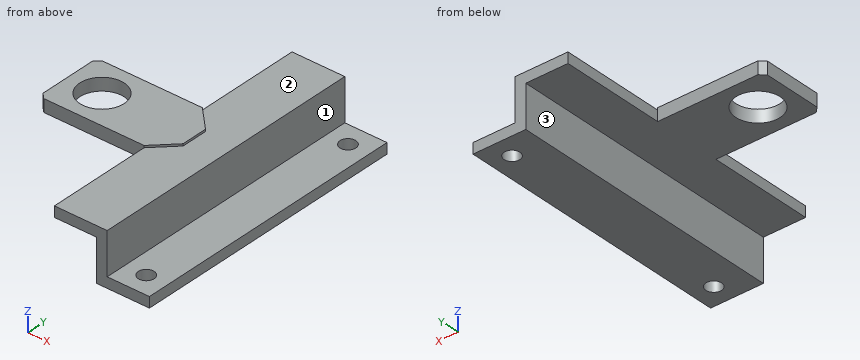
```python
from build123d import *

# Parameters (mm, degrees)
SKETCH_1_R          = 21
EXTRUDE_1_DEPTH     = 12
CHAMFER_1_SIZE      = 5
CHAMFER_2_SIZE      = 20
EXTRUDE_2_DEPTH     = 10
SKETCH_4_W          = 10
SKETCH_4_H          = 265
EXTRUDE_3_DEPTH     = 50
SKETCH_6_W          = 50
SKETCH_6_H          = 265
EXTRUDE_4_DEPTH     = 10
SKETCH_7_R          = 7.5
CUT_EXTRUDE_1_DEPTH = 211.063085762


with BuildPart() as part:
    # 草图1 → 凸台-拉伸1 (new body)
    with BuildSketch(Plane.XY):
        Polygon((32.5, 32.5), (87.5, 32.5), (87.5, -32.5), (32.5, -32.5), (-32.5, -32.5), (-32.5, 32.5), align=None)
        Circle(SKETCH_1_R, mode=Mode.SUBTRACT)
    extrude(amount=EXTRUDE_1_DEPTH)

    # 倒角1
    chamfer_1_edges = [part.edges().sort_by_distance(p)[0] for p in [
        (-32.5, -32.5, 6),
        (-32.5, 32.5, 6),
    ]]
    chamfer(chamfer_1_edges, length=CHAMFER_1_SIZE)

    # 倒角2
    chamfer_2_edges = [part.edges().sort_by_distance(p)[0] for p in [
        (87.5, 32.5, 6),
        (87.5, -32.5, 6),
    ]]
    chamfer(chamfer_2_edges, length=CHAMFER_2_SIZE)

    # 草图3 → 凸台-拉伸2 (add)
    with BuildSketch(Plane(origin=(0, 0, 0), x_dir=(-1, 0, 0), z_dir=(0, 0, -1))):
        Polygon((-67.5, 32.5), (-87.5, 12.5), (-87.5, -12.5), (-67.5, -32.5), (-67.5, -132.5), (-117.5, -132.5), (-117.5, 132.5), (-67.5, 132.5), align=None)
    extrude(amount=-EXTRUDE_2_DEPTH)

    # 草图4 → 凸台-拉伸3 (add)
    with BuildSketch(Plane.XY.offset(10)):
        with Locations((112.5, 0)):
            Rectangle(SKETCH_4_W, SKETCH_4_H)
    extrude(amount=-EXTRUDE_3_DEPTH)

    # 草图6 → 凸台-拉伸4 (add)
    with BuildSketch(Plane(origin=(0, 0, -40), x_dir=(-1, 0, 0), z_dir=(0, 0, -1))):
        with Locations((-132.5, 0)):
            Rectangle(SKETCH_6_W, SKETCH_6_H)
    extrude(amount=-EXTRUDE_4_DEPTH)

    # 草图7 → 切除-拉伸1 (cut, through all)
    with BuildSketch(Plane.XY.offset(-30)):
        with Locations((137.5, 112.5)):
            Circle(SKETCH_7_R)
        with Locations((137.5, -112.5)):
            Circle(SKETCH_7_R)
    extrude(amount=-CUT_EXTRUDE_1_DEPTH, mode=Mode.SUBTRACT)


solid = part.part
```
The listing builds one solid part. Answer for the finished solid, in the listing's coordinates (mm). Face numbers are marked on the shaded views. A direction names the side the tool comes from. Round coordinates to 2 decimals unless told otherwise and drop trailing zeros. Order: outer loops, then holes, each group sorted by start corner. A loop starts at its lowest first (then second) coordinate and runs counter-clockwise, first axis right, second up. Notation, with made-up numbers: (61, 49.25) - (68, 49.25) arc R4 cw to (68, 56.25) - close; hole circle Ø1 at (-22, 5.5). An arc over 180 degrees is marked (long way). Put each result on its own line as item: value. Start each with the question number.
(1) Find section A-A (y = 112.5). Give the vertices of the cut face in (x, z).
(2) Find section D-D (y = 0). Give the vertices of the cut face in (x, z), plus the area to 3 significant figures.
(3) Given P1, Ø6, axis at x = 31.5, z = 7, coming from the +Y side; P2, Ø12, axis at y = 96, z = -2.5, coming from the -X side; P3, Ø3.5, axis at x = 15.5, z = 6.5, coming from the -Y side; P4, Ø25, axis at x = 0, y = 0, coming from the -Z side, each flat-ended and moving along its own axis, determine where each tip first touches the part or whether it passes through.
(4) Find section C-C (x = 80). Give the vertices of the cut face in (y, z), plus the area to 3 significant figures.
(5) For the marked faces 1, 2 and 3, determine the directions among +Z, -Z, +X, -X, +Y, -Y from which every point of the face is accessible in a straight line to the end or side of a thin tool.
(6) Straight lines are drawn through the part: probe 1 along Y at (x, z) = (137, -32); probe 2 along Y at (x, z) = (0, 5); probe 3 along Z at (x, y) = (110.5, 117). For each, find the intervals that lie inside material, in ascending order. Write a range as from..to.
(7) Find section B-B (z = 7). Give the vertices of the cut face in (x, y).
Reply:
1. outline: (67.5, 0) - (107.5, 0) - (107.5, -40) - (130, -40) - (130, -30) - (117.5, -30) - (117.5, 10) - (67.5, 10) - close; (145, -40) - (157.5, -40) - (157.5, -30) - (145, -30) - close
2. outline: (-32.5, 0) - (-21, 0) - (-21, 12) - (-32.5, 12) - close; (21, 0) - (107.5, 0) - (107.5, -40) - (157.5, -40) - (157.5, -30) - (117.5, -30) - (117.5, 10) - (87.5, 10) - (87.5, 12) - (21, 12) - close
2. area: 2,040 mm^2
3. P1: y = 32.5
3. P2: x = 67.5
3. P3: y = -32.5
3. P4: through
4. outline: (-132.5, 0) - (132.5, 0) - (132.5, 10) - (20, 10) - (20, 12) - (-20, 12) - (-20, 10) - (-132.5, 10) - close
4. area: 2,730 mm^2
5. face 1: +Z, +X, +Y, -Y
5. face 2: +Z, +X
5. face 3: -Z, -X, +Y, -Y
6. probe 1: -132.5..-119.98, -105.02..105.02, 119.98..132.5
6. probe 2: -32.5..-21, 21..32.5
6. probe 3: -40..10
7. outline: (-32.5, -27.5) - (-27.5, -32.5) - (67.5, -32.5) - (67.5, -132.5) - (117.5, -132.5) - (117.5, 132.5) - (67.5, 132.5) - (67.5, 32.5) - (-27.5, 32.5) - (-32.5, 27.5) - close; hole circle Ø42 at (0, 0)
